```python
from build123d import *

# Parameters (mm, degrees)
SKETCH1_R                = 35
SKETCH1_R_2              = 15
BOSS_EXTRUDE2_DEPTH      = 767
SKETCH2_R                = 7.203487768
CUT_EXTRUDE1_DEPTH       = 767
PATTERN_CIRCULAR_1_COUNT = 16


with BuildPart() as part:
    # Sketch1 → Boss-Extrude2 (new body)
    with BuildSketch(Plane(origin=(0, 0, 0), x_dir=(0, 0, -1), z_dir=(1, 0, 0))):
        Circle(SKETCH1_R)
        Circle(SKETCH1_R_2, mode=Mode.SUBTRACT)
    extrude(amount=BOSS_EXTRUDE2_DEPTH)

    # Sketch2 → Cut-Extrude1 (cut)
    with BuildSketch(Plane.ZY):
        with Locations((0, 40.740922714)):
            Circle(SKETCH2_R)
    cut_extrude1 = extrude(amount=-CUT_EXTRUDE1_DEPTH, mode=Mode.SUBTRACT)

    # Pattern(Circular)1: Cut-Extrude1 ×16 about axis
    pattern_circular_1_axis = Axis((0, 0, 0), (1, 0, 0))
    for i in range(1, PATTERN_CIRCULAR_1_COUNT):
        add(cut_extrude1.rotate(pattern_circular_1_axis, i * 360 / PATTERN_CIRCULAR_1_COUNT), mode=Mode.SUBTRACT)


solid = part.part
```
Verification items for the finished model (mm, model axes). Give positions to 0.01 mm unless a question says otherwise; leave off trailing zeros. One line per item, written item: value.
(1) Gauge pin test, flat ends, axial feed: pin 1 (3 mm diameter, centred on x = 145.5, z = 17.5, fed in from +Y); pin 2 (8 mm diameter, centred on x = 321, y = 14, fed in from -Z); pin 3 (12 mm diameter, centred on y = 13, z = -3.5, fed in from +X); pin 4 (12 mm diameter, centred on x = 427.5, y = 22.5, fed in from +Z). Record the tip position at first contact, or that the pin passes through.
Final values:
pin 1: y = 30.58
pin 2: z = -33.1
pin 3: x = 767
pin 4: z = 30.58
(2) Draft check along Y on faces 1 (the face through (378.131, 0.66, 14.985)), 2 (the face through (0, -7, -15)). Enter one of: pulls with the +Y half, pulls with the -Y half, needs draft (parallel to the pull), parting line crosses it, or undercut.
Final values:
face 1: undercut
face 2: needs draft
(3) Scan lines: line 1 along Z through (x, y) = (690, -4); line 2 along Y through (x, z) = (347.5, 0); line 3 along Y through (x, z) = (384.5, -10). Record each from-to range of solid material in increasing order. Write a range as [from, to].
Final values:
line 1: [-34.75, -14.46], [14.46, 34.75]
line 2: [-33.54, -15], [15, 33.54]
line 3: [-33.1, -11.18], [11.18, 33.1]
